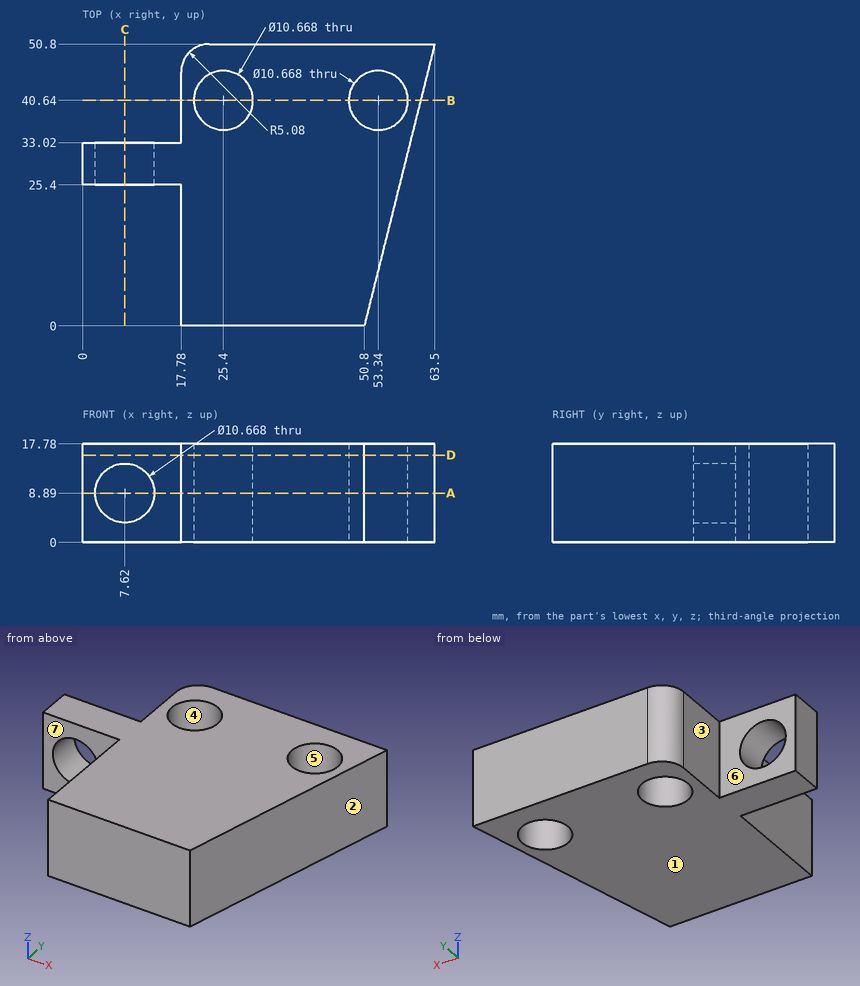
Part print with two shaded views. Sizes in mm from the minimum x, y, z corner. A direction names the side the tool comes from. Round coordinates to 2 decimals unless told otherwise and drop trailing zeros. Loops run counter-clockwise (first coordinate to the right, second up) from the corner with the lowest first, then second, coordinate; pieces in that order, holes last. Notation, with made-up numbers: M -23,6 L 20,6 A6 ccw 20,14 Z; hole C -20,-7.75 d8. An arc over 180 degrees is marked long. Return JSON: item names as keys, results as strings. Group by question number.
(1) Wall check: probe 1 along X at (y, z) = (38, 5.75); probe 2 along X at (y, z) = (45, 11.75); probe 3 along X at (y, z) = (30.75, 8.89). Give the ranges that are in metal, low to high. Write a range as [from, to].
(2) Drop flat-ended pins along their axis: P1, Ø10, axis at y = 37.5, z = 12, coming from the -X side; P2, Ø10, axis at x = 14, z = 13, coming from the +Y side; P3, Ø10, axis at y = 18.5, z = 15.5, coming from the +X side (3 decimals); P4, Ø9, axis at x = 6, z = 6, coming from the -Y side. Give the stop position or say it passes through.
(3) Saw through at B-B, the plane y = 40.64. List the corners of the cut face in (x, z), and give its area (3 significant figures).
(4) Saw through at A-A, the plane z = 8.89. List the corners of the cut face in (x, y), and give its area (3 significant figures).
(5) Saw through at D-D, the plane z = 15.75. List the corners of the cut face in (x, y), and give its area (3 significant figures).
(6) Mould opens along X. For the marked faces 1, 2, 3 and 4 say: +X half, -X half, draft (parallel to the pull), parting line (faces both ways), or undercut.
(7) Tool access for the marked faces 5, 6 and 7: list every direction of +Z, -Z, +X, -X, +Y, -Y with a clear straight run to the whole face (end or side of a thin tool).
(8) Saw through at C-C, the plane x = 7.62. List the corners of the cut face in (y, z).
Answer list:
{
 "1": {"probe 1": "[17.78, 20.77], [30.03, 48.71], [57.97, 60.3]", "probe 2": "[17.78, 22.33], [28.47, 50.27], [56.41, 62.05]", "probe 3": "[0, 2.29], [12.95, 58.49]"},
 "2": {"P1": "x = 0", "P2": "y = 49.02", "P3": "x = 56.675", "P4": "y = 25.4"},
 "3": {"outline": "M 17.78,0 L 20.07,0 L 20.07,17.78 L 17.78,17.78 Z; M 30.73,0 L 48.01,0 L 48.01,17.78 L 30.73,17.78 Z; M 58.67,0 L 60.96,0 L 60.96,17.78 L 58.67,17.78 Z", "area": "388 mm2"},
 "4": {"outline": "M 0,25.4 L 2.29,25.4 L 2.29,33.02 L 0,33.02 Z; M 12.95,25.4 L 17.78,25.4 L 17.78,0 L 50.8,0 L 63.5,50.8 L 22.86,50.8 A5.08 ccw 17.78,45.72 L 17.78,33.02 L 12.95,33.02 Z; hole C 25.4,40.64 d10.67; hole C 53.34,40.64 d10.67", "area": "1,870 mm2"},
 "5": {"outline": "M 0,25.4 L 17.78,25.4 L 17.78,0 L 50.8,0 L 63.5,50.8 L 22.86,50.8 A5.08 ccw 17.78,45.72 L 17.78,33.02 L 0,33.02 Z; hole C 25.4,40.64 d10.67; hole C 53.34,40.64 d10.67", "area": "1,950 mm2"},
 "6": {"face 1": "draft", "face 2": "+X half", "face 3": "-X half", "face 4": "undercut"},
 "7": {"face 5": "+Z, -Z", "face 6": "+Z, -Z, -X, +Y", "face 7": "+Z, -Z, -X, -Y"},
 "8": {"outline": "M 25.4,0 L 33.02,0 L 33.02,3.56 L 25.4,3.56 Z; M 25.4,14.22 L 33.02,14.22 L 33.02,17.78 L 25.4,17.78 Z"}
}
